Check sheet for the modelled part. Datum: model origin and axes. Units: mm. A direction names the side the tool comes from. Coordinates: 2 decimals unless noted, no trailing zeros. Write each loop counter-clockwise with the first axis right and the second up, starting at its lowest first coordinate (ties: lowest second). Pieces come first, ordered by that corner, then holes. Notation, with made-up numbers: (30, 56) - (35, 56) arc R9 cw to (35, 65) - close; hole circle Ø2 at (39, 55). An arc over 180 degrees is marked (long way). Answer as CSV lines item,"result". Start each with the question number.
from build123d import *

# Parameters (mm, degrees)
SKETCH_1_W          = 91
SKETCH_1_H          = 80
EXTRUDE_1_DEPTH     = 19
CUT_EXTRUDE_1_REACH = 73.514
SKETCH_2_W          = 30
SKETCH_2_H          = 65
FILLET_1_R          = 3


with BuildPart() as part:
    # 草图1 → 凸台-拉伸1 (new, symmetric)
    with BuildSketch(Plane.XY):
        Rectangle(SKETCH_1_W, SKETCH_1_H)
    extrude(amount=EXTRUDE_1_DEPTH, both=True)

    # 草图2 → 切除-拉伸1 (cut, up to next)
    with BuildSketch(Plane.XY.offset(19), mode=Mode.PRIVATE) as cut_extrude_1_sk1:
        with Locations((-30.5, -7.5)):
            Rectangle(SKETCH_2_W, SKETCH_2_H)
    cut_extrude_1_tool1 = extrude(cut_extrude_1_sk1.sketch, amount=-CUT_EXTRUDE_1_REACH, mode=Mode.PRIVATE) & part.part
    # 草图2 → 切除-拉伸1 (cut, up to next)
    with BuildSketch(Plane.XY.offset(19), mode=Mode.PRIVATE) as cut_extrude_1_sk2:
        with Locations((30.5, -7.5)):
            Rectangle(SKETCH_2_W, SKETCH_2_H)
    cut_extrude_1_tool2 = extrude(cut_extrude_1_sk2.sketch, amount=-CUT_EXTRUDE_1_REACH, mode=Mode.PRIVATE) & part.part
    add(cut_extrude_1_tool1.solids().sort_by_distance((-30.5, -7.5, 19))[0], mode=Mode.SUBTRACT)
    add(cut_extrude_1_tool2.solids().sort_by_distance((30.5, -7.5, 19))[0], mode=Mode.SUBTRACT)

    # 圆角1
    fillet_1_edges = [part.edges().sort_by_distance(p)[0] for p in [
        (-15.5, 25, 0),
        (15.5, 25, 0),
    ]]
    fillet(fillet_1_edges, radius=FILLET_1_R)


solid = part.part
(1) Cross-section at A-A on z = 0.5. Record the boundary of the cut face in (x, y).
(2) Cross-section at C-C on y = -5. Record the boundary of the cut face in (x, z).
(3) Release check for a two-part mould opening along X. For faces 1 (the face through (-32, 25, 0)), 2 (the face through (-16.4, 24.14, -0.27)), 3 (the face through (16.4, 24.14, -0.27)) record: pulls with the +X half, pulls with the -X half, needs draft (parallel to the pull), parting line crosses it, or undercut.
(4) Go/stop test with a flat-tipped pin: P1, Ø6, axis at y = 11.5, z = -9.5, coming from the -X side. Record where the tip stops, or that it passes through.
(5) Material ranges on probe 1 along X at (y, z) = (19, 14); probe 2 along Y at (x, z) = (35.5, 2), recorded low to high. Write a range as from..to.
(6) Cross-section at B-B on x = 23. Record the boundary of the cut face in (y, z), plus the area to 3 significant figures.
(7) Tool access check on faces 4 (the face through (-1, 40, 0)), 5 (the face through (-15.5, -9, 0)), 6 (the face through (32, 25, 0)). Record the directions out of +Z, -Z, +X, -X, +Y, -Y that give a thin tool (end or side, any length) a straight path to the whole face; none if there is none.
Checked values:
1,outline,"(-45.5, 25) - (-18.5, 25) arc R3 cw to (-15.5, 22) - (-15.5, -40) - (15.5, -40) - (15.5, 22) arc R3 cw to (18.5, 25) - (45.5, 25) - (45.5, 40) - (-45.5, 40) - close"
2,outline,"(-15.5, -19) - (15.5, -19) - (15.5, 19) - (-15.5, 19) - close"
3,face 1,"needs draft"
3,face 2,"pulls with the -X half"
3,face 3,"pulls with the +X half"
4,P1,"x = -15.5"
5,probe 1,"-15.5..15.5"
5,probe 2,"25..40"
6,outline,"(25, -19) - (40, -19) - (40, 19) - (25, 19) - close"
6,area,"570 mm^2"
7,face 4,"+Z, -Z, +X, -X, +Y"
7,face 5,"+Z, -Z, -X, -Y"
7,face 6,"+Z, -Z, +X, -Y"
